from build123d import *

# Parameters (mm, degrees)
EXTRUDE_1_DEPTH         = 13
HOLE_WIZARD_6_2_6_2_1_D = 6.2
SKETCH_4_R              = 27.5
CUT_EXTRUDE_1_DEPTH     = 8
CUT_EXTRUDE_2_REACH     = 54.934
SKETCH_5_R              = 22.5
CHAMFER_1_SIZE          = 2


with BuildPart() as part:
    # 草图1 → 凸台-拉伸1 (new body)
    with BuildSketch(Plane.XY):
        with BuildLine():
            Line((37, 0), (-37, 0))
            ThreePointArc((-37, 0), (-36.475571993, -6.2074671), (-34.917154173, -12.238968276))
            ThreePointArc((-34.917154173, -12.238968276), (-34.283867545, -17.214225736), (-35.739390486, -22.013776935))
            ThreePointArc((-35.739390486, -22.013776935), (-35.59944978, -32.031235087), (-26.9, -37))
            Line((-26.9, -37), (26.9, -37))
            ThreePointArc((26.9, -37), (35.59944978, -32.031235087), (35.739390486, -22.013776935))
            ThreePointArc((35.739390486, -22.013776935), (34.283867545, -17.214225736), (34.917154173, -12.238968276))
            ThreePointArc((34.917154173, -12.238968276), (36.475571993, -6.2074671), (37, 0))
        make_face()
        with BuildLine():
            Line((26.9, 37), (-26.9, 37))
            ThreePointArc((-26.9, 37), (-35.59944978, 32.031235087), (-35.739390486, 22.013776935))
            ThreePointArc((-35.739390486, 22.013776935), (-34.283867545, 17.214225736), (-34.917154173, 12.238968276))
            ThreePointArc((-34.917154173, 12.238968276), (-36.475571993, 6.2074671), (-37, 0))
            Line((-37, 0), (37, 0))
            ThreePointArc((37, 0), (36.475571993, 6.2074671), (34.917154173, 12.238968276))
            ThreePointArc((34.917154173, 12.238968276), (34.283867545, 17.214225736), (35.739390486, 22.013776935))
            ThreePointArc((35.739390486, 22.013776935), (35.59944978, 32.031235087), (26.9, 37))
        make_face()
    extrude(amount=EXTRUDE_1_DEPTH)

    # Ø6.2 (6.2) 直径孔1 (through all)
    with Locations(Plane(origin=(-26.870057685, 26.870057685, 13), x_dir=(1, 0, 0), z_dir=(0, 0, 1))):
        with Locations((0, 0), (53.74011537, 0), (53.74011537, -53.74011537), (0, -53.74011537)):
            Hole(HOLE_WIZARD_6_2_6_2_1_D / 2)

    # 草图4 → 切除-拉伸1 (cut)
    with BuildSketch(Plane.XY.offset(13)):
        Circle(SKETCH_4_R)
    extrude(amount=-CUT_EXTRUDE_1_DEPTH, mode=Mode.SUBTRACT)

    # 草图5 → 切除-拉伸2 (cut, up to next)
    with BuildSketch(Plane.XY.offset(5), mode=Mode.PRIVATE) as cut_extrude_2_sk1:
        Circle(SKETCH_5_R)
    cut_extrude_2_tool1 = extrude(cut_extrude_2_sk1.sketch, amount=-CUT_EXTRUDE_2_REACH, mode=Mode.PRIVATE) & part.part
    add(cut_extrude_2_tool1.solids().sort_by_distance((0, 0, 5))[0], mode=Mode.SUBTRACT)

    # 倒角1
    chamfer_1_edges = [part.edges().sort_by_distance(p)[0] for p in [
        (-22.5, 0, 0),
    ]]
    chamfer(chamfer_1_edges, length=CHAMFER_1_SIZE)


solid = part.part
Verification items for the finished model (mm, model axes). A direction names the side the tool comes from. Coordinates: 2 decimals unless noted, no trailing zeros. Loops run counter-clockwise (first coordinate to the right, second up) from the corner with the lowest first, then second, coordinate; pieces in that order, holes last. Notation, with made-up numbers: (6.25, 7) -> (54.25, 7) arc R31 ccw to (54.25, 40) -> close; hole circle Ø6 at (88, 0). An arc over 180 degrees is marked (long way). Answer as CSV lines item,"result".
1) Cross-section at D-D, the plane z = 7. Record the cut outline in (x, y), then the cut area to 3 significant figures.
Found:
outline,"(-35.74, -22.01) arc R10.1 ccw to (-26.9, -37) -> (26.9, -37) arc R10.1 ccw to (35.74, -22.01) arc R12 cw to (34.92, -12.24) arc R37 ccw to (34.92, 12.24) arc R12 cw to (35.74, 22.01) arc R10.1 ccw to (26.9, 37) -> (-26.9, 37) arc R10.1 ccw to (-35.74, 22.01) arc R12 cw to (-34.92, 12.24) arc R37 ccw to (-34.92, -12.24) arc R12 cw to start; hole circle Ø6.2 at (-26.87, -26.87); hole circle Ø6.2 at (-26.87, 26.87); hole circle Ø55 at (0, 0); hole circle Ø6.2 at (26.87, -26.87); hole circle Ø6.2 at (26.87, 26.87)"
area,"2,760 mm2"
2) Cross-section at B-B, the plane y = -28.5. Record the cut outline in (x, z).
Found:
outline,"(-36.87, 0) -> (-29.51, 0) -> (-29.51, 13) -> (-36.87, 13) -> close; (-24.23, 0) -> (24.23, 0) -> (24.23, 13) -> (-24.23, 13) -> close; (29.51, 0) -> (36.87, 0) -> (36.87, 13) -> (29.51, 13) -> close"
3) Cross-section at A-A, the plane x = 0. Record the cut outline in (y, z), then the cut area to 3 significant figures.
Found:
outline,"(-37, 0) -> (-24.5, 0) -> (-22.5, 2) -> (-22.5, 5) -> (-27.5, 5) -> (-27.5, 13) -> (-37, 13) -> close; (22.5, 2) -> (24.5, 0) -> (37, 0) -> (37, 13) -> (27.5, 13) -> (27.5, 5) -> (22.5, 5) -> close"
area,"293 mm2"
4) Release check for a two-part mould opening along X. For faces 3 (the cylindrical face through (-29.734, 25.683, 6.409)), 4 (the cylindrical face through (34.29, -17.28, 6.41)), 5 (the cylindrical face through (-35.673, -31.904, 6.409)) record: +X half, -X half, draft (parallel to the pull), parting line (faces both ways), or undercut.
Found:
face 3,"undercut"
face 4,"+X half"
face 5,"-X half"
5) Depth check by flat-ended pin: pin 1 (16.5 mm diameter, centred on x = -5, y = -10, fed in from +Z); pin 2 (3 mm diameter, centred on y = -2, z = 2, fed in from -X). Enter the tip coordinate at first touch or a pass-through.
Found:
pin 1,"passes through"
pin 2,"stops at x = -37"
6) Cross-section at C-C, the plane x = -26. Record the cut outline in (y, z), then the cut area to 3 significant figures.
Found:
outline,"(-37, 0) -> (-29.85, 0) -> (-29.85, 13) -> (-37, 13) -> close; (-23.89, 0) -> (23.89, 0) -> (23.89, 13) -> (8.96, 13) -> (8.96, 5) -> (-8.96, 5) -> (-8.96, 13) -> (-23.89, 13) -> close; (29.85, 0) -> (37, 0) -> (37, 13) -> (29.85, 13) -> close"
area,"664 mm2"
7) Thickness scan on L1, parallel to X at y = 16.5, z = 9.5; L2, parallel to X at y = -0.5, z = 4.75; L3, parallel to X at y = -29, z = 10.5. Record the ranges inside material, lowest first. Write a range as from..to.
Found:
L1,"x = -34.25..-22, 22..34.25"
L2,"x = -37..-22.49, 22.49..37"
L3,"x = -36.78..-29.12, -24.62..24.62, 29.12..36.78"
8) Tool access check on faces 1 (the cylindrical face through (23.913, -25.939, 6.409)), 2 (the flat face through (-23, 0, 5)). Record the directions out of +Z, -Z, +X, -X, +Y, -Y that give a thin tool (end or side, any length) a straight path to the whole face; none if there is none.
Found:
face 1,"+Z, -Z"
face 2,"+Z"
